from build123d import *

# Parameters (mm, degrees)
BOSS_EXTRUDE1_DEPTH      = 20
BOSS_EXTRUDE1_DEPTH_BACK = 20
SKETCH2_R                = 2.5
CUT_EXTRUDE1_DEPTH       = 20
FILLET1_R                = 1


with BuildPart() as part:
    # Sketch1 → Boss-Extrude1 (new, two sides: drawn at the far end of the back side and taken through both)
    with BuildSketch(Plane.XY.offset(-BOSS_EXTRUDE1_DEPTH_BACK)):
        with BuildLine():
            Line((-47.5, 0), (-30.945362405, 0))
            ThreePointArc((-30.945362405, 0), (-30.53852382, 0.086499937), (-30.202068258, 0.331035268))
            Line((-30.202068258, 0.331035268), (-26.297931742, 4.668964732))
            ThreePointArc((-26.297931742, 4.668964732), (-25.96147618, 4.913500063), (-25.554637595, 5))
            Line((-25.554637595, 5), (25.554637595, 5))
            ThreePointArc((25.554637595, 5), (25.96147618, 4.913500063), (26.297931742, 4.668964732))
            Line((26.297931742, 4.668964732), (30.202068258, 0.331035268))
            ThreePointArc((30.202068258, 0.331035268), (30.53852382, 0.086499937), (30.945362405, 0))
            Line((30.945362405, 0), (47.5, 0))
            Line((47.5, 0), (47.5, -2))
            Line((47.5, -2), (30.054637595, -2))
            ThreePointArc((30.054637595, -2), (29.64779901, -1.913500063), (29.311343449, -1.668964732))
            Line((29.311343449, -1.668964732), (25.407206932, 2.668964732))
            ThreePointArc((25.407206932, 2.668964732), (25.070751371, 2.913500063), (24.663912786, 3))
            Line((24.663912786, 3), (-24.663912786, 3))
            ThreePointArc((-24.663912786, 3), (-25.070751371, 2.913500063), (-25.407206932, 2.668964732))
            Line((-25.407206932, 2.668964732), (-29.311343449, -1.668964732))
            ThreePointArc((-29.311343449, -1.668964732), (-29.64779901, -1.913500063), (-30.054637595, -2))
            Line((-30.054637595, -2), (-47.5, -2))
            Line((-47.5, -2), (-47.5, 0))
        make_face()
    extrude(amount=BOSS_EXTRUDE1_DEPTH + BOSS_EXTRUDE1_DEPTH_BACK)

    # Sketch2 → Cut-Extrude1 (cut)
    with BuildSketch(Plane(origin=(0, 0, 0), x_dir=(1, 0, 0), z_dir=(0, 1, 0))):
        with Locations(Location((-38, 15, 0), (0, 0, 180))):
            Circle(SKETCH2_R)
        with Locations(Location((38, 15, 0), (0, 0, 90))):
            Circle(SKETCH2_R)
        with Locations(Location((38, -15, 0), (0, 0, 180))):
            Circle(SKETCH2_R)
        with Locations(Location((-38, -15, 0), (0, 0, 90))):
            Circle(SKETCH2_R)
    extrude(amount=-CUT_EXTRUDE1_DEPTH, mode=Mode.SUBTRACT)

    # Fillet1
    fillet1_edges = [part.edges().sort_by_distance(p)[0] for p in [
        (47.5, -1, -20),
        (-47.5, -1, -20),
        (-47.5, -1, 20),
        (47.5, -1, 20),
    ]]
    fillet(fillet1_edges, radius=FILLET1_R)


solid = part.part
Work out the finished part from the listing and answer in its coordinate system (mm). A direction names the side the tool comes from. Coordinates: 2 decimals unless noted, no trailing zeros. Loops run counter-clockwise (first coordinate to the right, second up) from the corner with the lowest first, then second, coordinate; pieces in that order, holes last. Notation, with made-up numbers: M 23,30 L 79,30 A10 ccw 79,44 Z; hole C 58.25,19.5 d2. An arc over 180 degrees is marked long. Answer in a Markdown table with one row per item. Add a question column.
1. Find section B-B, the plane z = -15. Write down the section's boundary in (x, y), then the cut area to 3 significant figures.
2. Flat-ended cylindrical pins translate along their axes: P1, Ø3, axis at x = 30.5, y = 3, coming from the -Z side; P2, Ø18, axis at x = -35.5, z = -2, coming from the +Y side; P3, Ø1.5, axis at x = -13, z = 4.5, coming from the -Y side; P4, Ø1.5, axis at y = 2.5, z = 11, coming from the -X side (3 decimals). Find the tip coordinate at first contact, or state that the pin passes through.
3. The mould has two halves that part along X. Classify faces 6 (the cylindrical face through (-40.31, -0.99, -15.96)), 7 (the flat face through (-28.277, 2.47, -0.28)), 8 (the flat face through (0, 5, 0)), 9 (the cylindrical face through (35.69, -0.99, 14.04)): pulls with the +X half, pulls with the -X half, needs draft (parallel to the pull), parting line crosses it, or undercut.
4. Find section C-C, the plane y = 1.5. Write down the section's boundary in (x, z), then the cut area to 3 significant figures.
5. Find section A-A, the plane x = -38. Write down the section's boundary in (y, z), then the cut area to 3 significant figures.
6. Find section D-D, the plane z = -5. Write down the section's boundary in (x, y).
7. A tool of negligible diameter and unlimited length cuts with its end or side. For faces 1 (the flat face through (39, -2, 0)), 2 (the cylindrical face through (-35.56, -0.99, 15.54)), 3 (the flat face through (39, 0, 0)), 4 (the flat face through (-39, 0, 0)), 5 (the flat face through (27.387, 0.47, -0.28)), from which of +Z, -Z, +X, -X, +Y, -Y can it reach the whole face along a straight path? Write none if from no direction.
8. Consider L1, parallel to Z at x = -38, y = -1.15; L2, parallel to Y at x = 32.5, z = 3.5; L3, parallel to X at y = 1, z = 15.5. Determine where each line is inside the solid, lowest interval first.
Reported:
| question | item | result |
|---|---|---|
| 1 | outline | M -47.5,-2 L -40.5,-2 L -40.5,0 L -47.5,0 Z; M -35.5,-2 L -30.05,-2 A1 ccw -29.31,-1.67 L -25.41,2.67 A1 cw -24.66,3 L 24.66,3 A1 cw 25.41,2.67 L 29.31,-1.67 A1 ccw 30.05,-2 L 35.5,-2 L 35.5,0 L 30.95,0 A1 cw 30.2,0.33 L 26.3,4.67 A1 ccw 25.55,5 L -25.55,5 A1 ccw -26.3,4.67 L -30.2,0.33 A1 cw -30.95,0 L -35.5,0 Z; M 40.5,-2 L 47.5,-2 L 47.5,0 L 40.5,0 Z |
| 1 | area | 179 mm^2 |
| 2 | P1 | passes through |
| 2 | P2 | stops at y = 4.44 |
| 2 | P3 | stops at y = 3 |
| 2 | P4 | stops at x = -28.925 |
| 3 | face 6 | undercut |
| 3 | face 7 | pulls with the -X half |
| 3 | face 8 | needs draft |
| 3 | face 9 | undercut |
| 4 | outline | M -29.15,-20 L -26.46,-20 L -26.46,20 L -29.15,20 Z; M 26.46,-20 L 29.15,-20 L 29.15,20 L 26.46,20 Z |
| 4 | area | 215 mm^2 |
| 5 | outline | M -2,-20 L 0,-20 L 0,-17.5 L -2,-17.5 Z; M -2,-12.5 L 0,-12.5 L 0,12.5 L -2,12.5 Z; M -2,17.5 L 0,17.5 L 0,20 L -2,20 Z |
| 5 | area | 60.0 mm^2 |
| 6 | outline | M -47.5,-2 L -30.05,-2 A1 ccw -29.31,-1.67 L -25.41,2.67 A1 cw -24.66,3 L 24.66,3 A1 cw 25.41,2.67 L 29.31,-1.67 A1 ccw 30.05,-2 L 47.5,-2 L 47.5,0 L 30.95,0 A1 cw 30.2,0.33 L 26.3,4.67 A1 ccw 25.55,5 L -25.55,5 A1 ccw -26.3,4.67 L -30.2,0.33 A1 cw -30.95,0 L -47.5,0 Z |
| 7 | face 1 | +Z, -Z, +X, -X, -Y |
| 7 | face 2 | +Y, -Y |
| 7 | face 3 | +Z, -Z, +X, +Y |
| 7 | face 4 | +Z, -Z, -X, +Y |
| 7 | face 5 | +Z, -Z, -Y |
| 8 | L1 | z = -20 to -17.5, -12.5 to 12.5, 17.5 to 20 |
| 8 | L2 | y = -2 to 0 |
| 8 | L3 | x = -29.6 to -26.91, 26.91 to 29.6 |
